Model file for the job. Use its own axes, mm. Give positions to 0.01 mm unless a question says otherwise; leave off trailing zeros. Write each loop counter-clockwise with the first axis right and the second up, starting at its lowest first coordinate (ties: lowest second). Pieces come first, ordered by that corner, then holes. Notation, with made-up numbers: (27, 63) - (79, 63) arc R4 cw to (79, 70) - close; hole circle Ø10 at (33.5, 84). An arc over 180 degrees is marked (long way). One line per item, written item: value. Start each with the question number.
(1) Mould opens along X. For faces 1 (the face through (-9.86, 0.986, 37.535)), 2 (the face through (-9.5, 1, -18)), 3 (the face through (0, 2, -1)) say: pulls with the +X half, pulls with the -X half, needs draft (parallel to the pull), parting line crosses it, or undercut.
(2) Cut at A-A, the plane x = 8. List the corners of the cut face in (y, z), and give its area (3 significant figures).
(3) Probe L1, parallel to X at y = 1.15, z = -20; L2, parallel to Z at x = -7, y = 0.15; L3, parallel to Z at x = -14, y = 0.95. List the from-to ranges inside material, lowest first.
(4) Drop flat-ended pins along their axis: P1, Ø4.5, axis at x = 8, z = -20, coming from the -Y side; P2, Ø3, axis at x = -10, z = 16, coming from the -Y side. Give the stop position or say it passes through.
(5) Cut at C-C, the plane y = 1.6. List the corners of the cut face in (x, z).
(6) Cut at D-D, the plane x = -8. List the corners of the cut face in (y, z), and give its area (3 significant figures).
(7) Cut at B-B, the plane z = -20. List the corners of the cut face in (x, y), and give its area (3 significant figures).
from build123d import *
from OCP.BRepFilletAPI import BRepFilletAPI_MakeChamfer

# Parameters (mm, degrees)
SKETCH1_W           = 40
SKETCH1_H           = 80
BOSS_EXTRUDE1_DEPTH = 2
SKETCH2_R           = 2.5
CUT_EXTRUDE1_DEPTH  = 10
CHAMFER1_SIZE       = 5
CHAMFER1_SIZE2      = 20


with BuildPart() as part:
    # Sketch1 → Boss-Extrude1 (new body)
    with BuildSketch(Plane(origin=(0, 0, 0), x_dir=(1, 0, 0), z_dir=(0, 1, 0))):
        Rectangle(SKETCH1_W, SKETCH1_H)
    extrude(amount=BOSS_EXTRUDE1_DEPTH)

    # Sketch2 → Cut-Extrude1 (cut)
    with BuildSketch(Plane.XZ):
        with Locations(Location((8, -20, 0), (0, 0, 270))):
            Circle(SKETCH2_R)
        with Locations(Location((-8, -20, 0), (0, 0, 270))):
            Circle(SKETCH2_R)
    extrude(amount=-CUT_EXTRUDE1_DEPTH, mode=Mode.SUBTRACT)

    # Chamfer1: one chamfer whose edges measure the first distance from different faces: ONE call of the kernel's chamfer builder (chamfer() names one face for all edges)
    chamfer1_edges_1 = [part.edges().sort_by_distance(p)[0] for p in [
        (20, 1, 40),
    ]]
    chamfer1_side_1 = [part.faces().sort_by_distance(p)[0] for p in [
        (0, 1, 40),
    ]]
    chamfer1_edges_2 = [part.edges().sort_by_distance(p)[0] for p in [
        (-20, 1, 40),
    ]]
    chamfer1_side_2 = [part.faces().sort_by_distance(p)[0] for p in [
        (-20, 1, 0),
    ]]
    chamfer1 = BRepFilletAPI_MakeChamfer(part.part.solid().wrapped)
    for e in chamfer1_edges_1:
        chamfer1.Add(CHAMFER1_SIZE, CHAMFER1_SIZE2, e.wrapped, chamfer1_side_1[0].wrapped)  # the first distance lies on this face
    for e in chamfer1_edges_2:
        chamfer1.Add(CHAMFER1_SIZE, CHAMFER1_SIZE2, e.wrapped, chamfer1_side_2[0].wrapped)  # the first distance lies on this face
    add(Compound.cast(chamfer1.Shape()), mode=Mode.REPLACE)


solid = part.part
Answers follow:
1. face 1: pulls with the -X half
1. face 2: undercut
1. face 3: needs draft
2. outline: (0, -40) - (2, -40) - (2, -22.5) - (0, -22.5) - close; (0, -17.5) - (2, -17.5) - (2, 40) - (0, 40) - close
2. area: 150 mm²
3. L1: x = -20 to -10.5, -5.5 to 5.5, 10.5 to 20
3. L2: z = -40 to -22.29, -17.71 to 38.25
3. L3: z = -40 to 36.5
4. P1: passes through
4. P2: stops at y = 0
5. outline: (-20, -40) - (20, -40) - (20, 20) - (15, 40) - (0, 40) - (-20, 35) - close; hole circle Ø5 at (-8, -20); hole circle Ø5 at (8, -20)
6. outline: (0, -40) - (2, -40) - (2, -22.5) - (0, -22.5) - close; (0, -17.5) - (2, -17.5) - (2, 38) - (0, 38) - close
6. area: 146 mm²
7. outline: (-20, 0) - (-10.5, 0) - (-10.5, 2) - (-20, 2) - close; (-5.5, 0) - (5.5, 0) - (5.5, 2) - (-5.5, 2) - close; (10.5, 0) - (20, 0) - (20, 2) - (10.5, 2) - close
7. area: 60.0 mm²
